```python
from build123d import *

# Parameters (mm, degrees)
SKETCH1_R               = 2
BOSS_EXTRUDE1_DEPTH     = 8.2
M2_5_TAPPED_HOLE1_D     = 2.05
M2_5_TAPPED_HOLE1_DEPTH = 6.35
M2_5_TAPPED_HOLE1_TIP   = 0.615882135
SKETCH8_R               = 3
BOSS_EXTRUDE2_DEPTH     = 3
CHAMFER1_SIZE           = 0.2
CHAMFER2_SIZE           = 0.2


with BuildPart() as part:
    # Sketch1 → Boss-Extrude1 (new body)
    with BuildSketch(Plane(origin=(0, 0, 0), x_dir=(1, 0, 0), z_dir=(0, 1, 0))):
        with Locations(Location((0, 0, 0), (0, 0, 270))):
            Circle(SKETCH1_R)
    extrude(amount=BOSS_EXTRUDE1_DEPTH)

    # M2.5 Tapped Hole1
    with Locations(Plane(origin=(0, 8.2, 0), x_dir=(1, 0, 0), z_dir=(0, 1, 0))):
        with Locations((0, 0.004175621)):
            Hole(M2_5_TAPPED_HOLE1_D / 2, depth=M2_5_TAPPED_HOLE1_DEPTH)
            with Locations((0, 0, -(M2_5_TAPPED_HOLE1_DEPTH + M2_5_TAPPED_HOLE1_TIP / 2))):  # 118° drill point
                Cone(0, M2_5_TAPPED_HOLE1_D / 2, M2_5_TAPPED_HOLE1_TIP, mode=Mode.SUBTRACT)

    # Sketch8 → Boss-Extrude2 (add)
    with BuildSketch(Plane.XZ):
        with Locations(Location((0, 0, 0), (0, 0, 270))):
            Circle(SKETCH8_R)
    extrude(amount=-BOSS_EXTRUDE2_DEPTH)

    # Chamfer1
    chamfer1_edges = [part.edges().sort_by_distance(p)[0] for p in [
        (0, 8.2, -2),
    ]]
    chamfer(chamfer1_edges, length=CHAMFER1_SIZE)

    # Chamfer2
    chamfer2_edges = [part.edges().sort_by_distance(p)[0] for p in [
        (0, 0, 3),
        (0, 3, 3),
    ]]
    chamfer(chamfer2_edges, length=CHAMFER2_SIZE)


solid = part.part
```
Model file for the job. Use its own axes, mm. A direction names the side the tool comes from. Coordinates: 2 decimals unless noted, no trailing zeros. Order: outer loops, then holes, each group sorted by start corner. A loop starts at its lowest first (then second) coordinate and runs counter-clockwise, first axis right, second up. Notation, with made-up numbers: (16, -11) -> (22, -11) arc R14 ccw to (22, 14) -> close; hole circle Ø7 at (-32, -7.5). An arc over 180 degrees is marked (long way). Return JSON: item names as keys, results as strings.
Item 1: Slice it at C-C (y = 4.25). Write the cut outline in (x, z) (3 decimals), then the cut area to 3 significant figures.
Model answer:
{"outline": "circle Ø4 at (0, 0); hole circle Ø2.05 at (0, -0.004)", "area": "9.27 mm²"}
Item 2: Pin check, flat tips, straight feed: P1, Ø1, axis at x = 0.5, y = 5, coming from the -Z side; P2, Ø2.5, axis at x = 0, z = 0, coming from the +Y side; P3, Ø0.6, axis at x = 0, z = -0.5, coming from the +Y side; P4, Ø1.5, axis at y = 5, z = 1.5, coming from the -X side. Stop position of each tip, or through.
Model answer:
{"P1": "stops at z = -2", "P2": "stops at y = 8.2", "P3": "stops at y = 3", "P4": "stops at x = -1.85"}
Item 3: Wall check: line 1 along Z through (x, y) = (0, 4.5); line 2 along Y through (x, z) = (0.5, -2.7); line 3 along X through (y, z) = (3.5, 0.1). Give the ranges that are in metal, low to high. Write a range as from..to.
Model answer:
{"line 1": "z = -2..-1.03, 1.02..2", "line 2": "y = 0..3", "line 3": "x = -2..-1.02, 1.02..2"}
Item 4: 3-axis set-ups, long thin cutter, end or side, ignore diameter. For faces 1 (the face through (0, 3, 0)), 2 (the face through (0.9, 1.48, -2.86)): which of +Z, -Z, +X, -X, +Y, -Y reach the whole face in a straight line?
Model answer:
{"face 1": "+Y", "face 2": "+Y, -Y"}
Item 5: Slice it at B-B (y = 2.25). Write the cut outline in (x, z), then the cut area to 3 significant figures.
Model answer:
{"outline": "circle Ø6 at (0, 0)", "area": "28.3 mm²"}
Item 6: Slice it at A-A (x = 0). Write the cut outline in (y, z), then the cut area to 3 significant figures.
Model answer:
{"outline": "(0, -2.8) -> (0.2, -3) -> (2.8, -3) -> (3, -2.8) -> (3, -2) -> (8, -2) -> (8.2, -1.8) -> (8.2, -1.03) -> (3, -1.03) -> (3, 1.02) -> (8.2, 1.02) -> (8.2, 1.8) -> (8, 2) -> (3, 2) -> (3, 2.8) -> (2.8, 3) -> (0.2, 3) -> (0, 2.8) -> close", "area": "28.0 mm²"}
